Input: dimensioned drawing with shaded views. Units: mm. Origin: part minimum x, y, z. Round coordinates to 2 decimals unless told otherwise and drop trailing zeros. Loops run counter-clockwise (first coordinate to the right, second up) from the corner with the lowest first, then second, coordinate; pieces in that order, holes last. Notation, with made-up numbers: (53.5, 24.25) - (61.5, 24.25) arc R27 cw to (61.5, 52.25) - close; hole circle Ø5 at (76, 79.5). An arc over 180 degrees is marked (long way). Write each question's results on one line, items separated by ' | '.
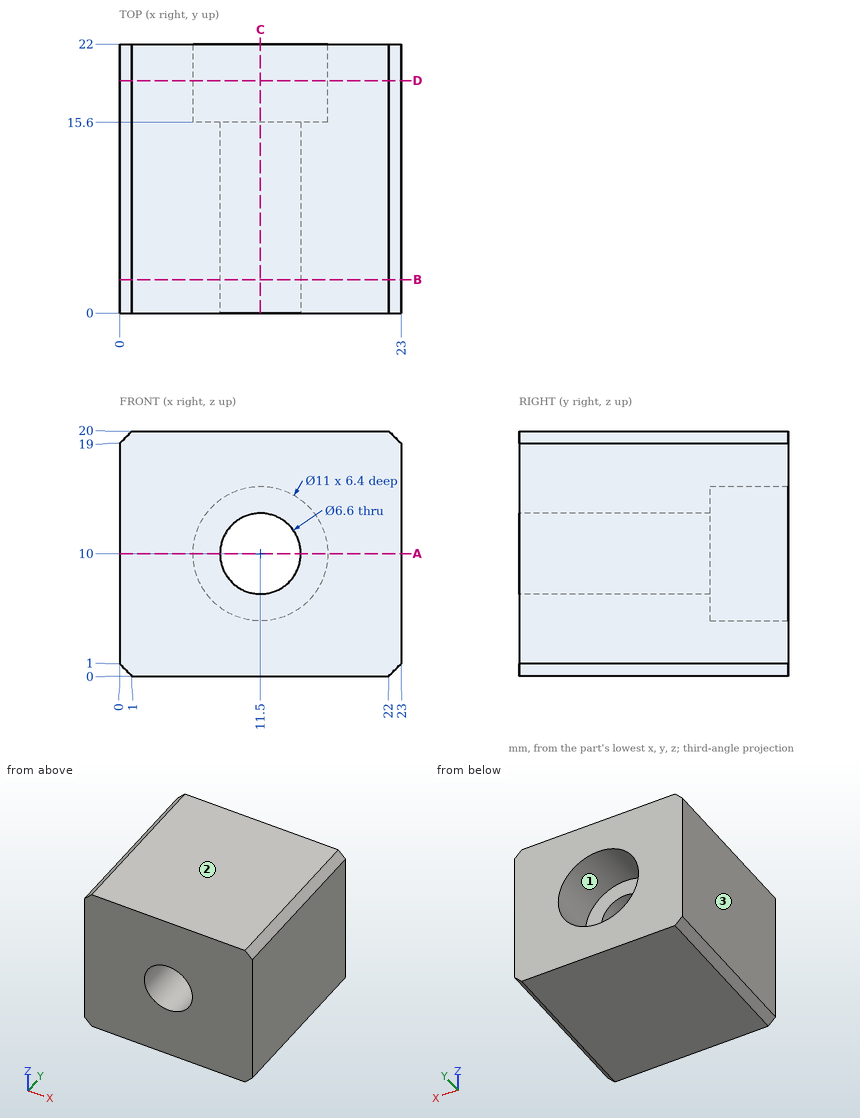
1. Section query A-A, the plane z = 10. Output: boundary loops of the cut face in (x, y), plus the area to 3 significant figures.
Answer:
outline: (0, 0) - (8.2, 0) - (8.2, 15.6) - (6, 15.6) - (6, 22) - (0, 22) - close; (14.8, 0) - (23, 0) - (23, 22) - (17, 22) - (17, 15.6) - (14.8, 15.6) - close | area: 333 mm^2
2. Line query: line 1 (Z direction, x = 11.5, y = 19.5); line 2 (Z direction, x = 11.5, y = 7); line 3 (Y direction, x = 7.75, z = 9.5). Output: solid intervals per line, ascending. Write a range as [from, to].
Answer:
line 1: [0, 4.5], [15.5, 20] | line 2: [0, 6.7], [13.3, 20] | line 3: [0, 15.6]
3. Mould query, pull axis X, two halves, no side actions, for the marked faces 1, 2 and 3. Classes: pulls with the +X half, pulls with the -X half, needs draft (parallel to the pull), parting line crosses it, or undercut.
Answer:
face 1: undercut | face 2: needs draft | face 3: pulls with the -X half
4. Section query C-C, the plane x = 11.5. Output: boundary loops of the cut face in (y, z).
Answer:
outline: (0, 0) - (22, 0) - (22, 4.5) - (15.6, 4.5) - (15.6, 6.7) - (0, 6.7) - close; (0, 13.3) - (15.6, 13.3) - (15.6, 15.5) - (22, 15.5) - (22, 20) - (0, 20) - close
5. Section query D-D, the plane y = 19. Output: boundary loops of the cut face in (x, z).
Answer:
outline: (0, 1) - (1, 0) - (22, 0) - (23, 1) - (23, 19) - (22, 20) - (1, 20) - (0, 19) - close; hole circle Ø11 at (11.5, 10)
6. Section query B-B, the plane y = 2.75. Output: boundary loops of the cut face in (x, z), plus the area to 3 significant figures.
Answer:
outline: (0, 1) - (1, 0) - (22, 0) - (23, 1) - (23, 19) - (22, 20) - (1, 20) - (0, 19) - close; hole circle Ø6.6 at (11.5, 10) | area: 424 mm^2
7. Contact query for a flat-ended pin moving along its axis: pin 1 (6 mm diameter, centred on x = 11.5, z = 10, fed in from -Y). Output: stop coordinate, or through.
Answer:
pin 1: through
